Build history of the part. All positions in model axes, mm. Give positions to 0.01 mm unless a question says otherwise; leave off trailing zeros. Order: outer loops, then holes, each group sorted by start corner. A loop starts at its lowest first (then second) coordinate and runs counter-clockwise, first axis right, second up. Notation, with made-up numbers: (-40, 74) - (-18, 74) arc R26 cw to (-18, 95) - close; hole circle Ø6 at (-38, 89.25). An arc over 180 degrees is marked (long way). Answer in a Markdown table with one row per item.
```python
from build123d import *

# Parameters (mm, degrees)
SKETCH1_R           = 32
SKETCH1_R_2         = 20
BOSS_EXTRUDE1_DEPTH = 0.5
SKETCH2_R           = 2.5
CUT_EXTRUDE1_DEPTH  = 0.5


with BuildPart() as part:
    # Sketch1 → Boss-Extrude1 (new body)
    with BuildSketch(Plane.XY):
        Circle(SKETCH1_R)
        Circle(SKETCH1_R_2, mode=Mode.SUBTRACT)
    extrude(amount=BOSS_EXTRUDE1_DEPTH)

    # Sketch2 → Cut-Extrude1 (cut)
    with BuildSketch(Plane.XY.offset(0.5)):
        with Locations((0, 25)):
            Circle(SKETCH2_R)
        with Locations((21.650635095, -12.5)):
            Circle(SKETCH2_R)
        with Locations((-21.650635095, -12.5)):
            Circle(SKETCH2_R)
    extrude(amount=-CUT_EXTRUDE1_DEPTH, mode=Mode.SUBTRACT)


solid = part.part
```
1. Cut at C-C on z = 0.35. Write the cut outline in (x, y), and give its area (3 significant figures).
Check result:
| item | result |
|---|---|
| outline | circle Ø64 at (0, 0); hole circle Ø5 at (-21.65, -12.5); hole circle Ø40 at (0, 0); hole circle Ø5 at (0, 25); hole circle Ø5 at (21.65, -12.5) |
| area | 1,900 mm² |
2. Two-plate mould, pull along X, no slides. Class faces 1 (the face through (-4.336, -19.524, 0.246)), 2 (the face through (14, 15, 0.5)), 3 (the face through (-6.94, -31.24, 0.25)), 4 (the face through (-0.33, 27.48, 0.25)): +X half, -X half, draft (parallel to the pull), parting line (faces both ways), or undercut.
Check result:
| item | result |
|---|---|
| face 1 | undercut |
| face 2 | draft |
| face 3 | parting line |
| face 4 | undercut |
3. Cut at A-A on y = 0. Write the cut outline in (x, z).
Check result:
| item | result |
|---|---|
| outline | (-32, 0) - (-20, 0) - (-20, 0.5) - (-32, 0.5) - close; (20, 0) - (32, 0) - (32, 0.5) - (20, 0.5) - close |
4. Probe line 1 (Y direction, x = 0, z = 0.3); line 2 (X direction, y = 6.5, z = 0.1); line 3 (X direction, y = 8, z = 0.05). List the from-to ranges inside material, lowest first.
Check result:
| item | result |
|---|---|
| line 1 | y = -32 to -20, 20 to 22.5, 27.5 to 32 |
| line 2 | x = -31.33 to -18.91, 18.91 to 31.33 |
| line 3 | x = -30.98 to -18.33, 18.33 to 30.98 |
5. Cut at B-B on x = 0. Write the cut outline in (y, z).
Check result:
| item | result |
|---|---|
| outline | (-32, 0) - (-20, 0) - (-20, 0.5) - (-32, 0.5) - close; (20, 0) - (22.5, 0) - (22.5, 0.5) - (20, 0.5) - close; (27.5, 0) - (32, 0) - (32, 0.5) - (27.5, 0.5) - close |
6. Cut at D-D on y = -12.5. Write the cut outline in (x, z), and give its area (3 significant figures).
Check result:
| item | result |
|---|---|
| outline | (-29.46, 0) - (-24.15, 0) - (-24.15, 0.5) - (-29.46, 0.5) - close; (-19.15, 0) - (-15.61, 0) - (-15.61, 0.5) - (-19.15, 0.5) - close; (15.61, 0) - (19.15, 0) - (19.15, 0.5) - (15.61, 0.5) - close; (24.15, 0) - (29.46, 0) - (29.46, 0.5) - (24.15, 0.5) - close |
| area | 8.85 mm² |
